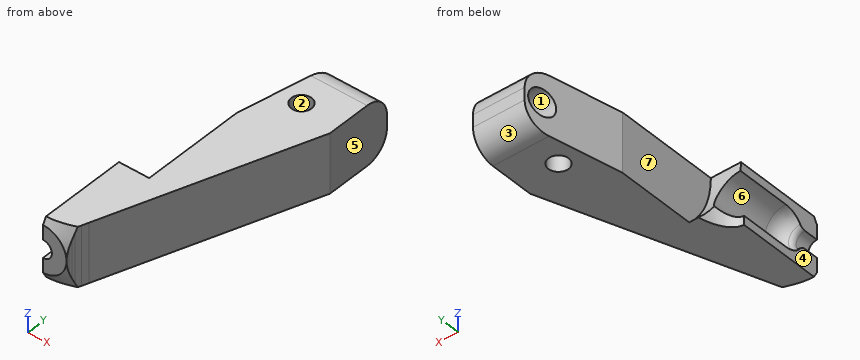
from build123d import *

# Parameters (mm, degrees)
SKETCH1_R                      = 3
BOSS_EXTRUDE2_DEPTH            = 17.7
CUT_EXTRUDE1_REACH             = 94.786
CUT_EXTRUDE1_DIRECTION_2_REACH = 94.786
SKETCH6_RX                     = 12.258033
SKETCH6_RY                     = 6.491927
CUT_EXTRUDE2_DEPTH             = 48.7
SKETCH7_R                      = 6.19409
CUT_EXTRUDE3_DEPTH             = 60.7
SKETCH8_R                      = 4
CUT_EXTRUDE4_DEPTH             = 48
FILLET1_R                      = 7
SKETCH10_OUTSIDE_W             = 249.546
SKETCH10_OUTSIDE_H             = 207.246
SKETCH10_OUTSIDE_R             = 7
CUT_EXTRUDE5_DEPTH             = 48
CUT_EXTRUDE5_TAPER             = 60
CUT_EXTRUDE8_DEPTH             = 44


with BuildPart() as part:
    # Sketch1 → Boss-Extrude2 (new body)
    with BuildSketch(Plane.XY):
        with BuildLine():
            Line((39, -51.503555), (34.837666, -51.503555))
            Line((34.837666, -51.503555), (25.162334, -51.503555))
            Line((25.162334, -51.503555), (21, -51.503555))
            Line((21, -51.503555), (21, -28.6))
            Line((21, -28.6), (15.376404, 0))
            Line((15.376404, 0), (0, 0))
            Line((0, 0), (0, -20.136364))
            Line((0, -20.136364), (21.048788, -80.412439))
            add(Edge.make_bspline(
                [(21.669142, -82.188906), (21.466678, -81.609123), (21.259066, -81.014599), (21.048788, -80.412439)],
                knots=[0.75, 0.75, 0.75, 0.75, 1, 1, 1, 1], degree=3))
            add(Edge.make_bspline(
                [(22.255532, -83.868113), (22.06924, -83.334643), (21.871606, -82.768689), (21.669142, -82.188906)],
                knots=[0.5, 0.5, 0.5, 0.5, 0.75, 0.75, 0.75, 0.75], degree=3))
            add(Edge.make_bspline(
                [(22.524034, -84.637007), (22.439154, -84.393941), (22.348677, -84.134848), (22.255532, -83.868113)],
                knots=[0.375, 0.375, 0.375, 0.375, 0.5, 0.5, 0.5, 0.5], degree=3))
            add(Edge.make_bspline(
                [(22.758263, -85.307753), (22.688292, -85.107381), (22.608914, -84.880073), (22.524034, -84.637007)],
                knots=[0.25, 0.25, 0.25, 0.25, 0.375, 0.375, 0.375, 0.375], degree=3))
            add(Edge.make_bspline(
                [(22.855261, -85.585519), (22.825847, -85.50129), (22.793248, -85.407938), (22.758263, -85.307753)],
                knots=[0.1875, 0.1875, 0.1875, 0.1875, 0.25, 0.25, 0.25, 0.25], degree=3))
            add(Edge.make_bspline(
                [(22.932474, -85.806631), (22.910958, -85.745015), (22.884674, -85.669748), (22.855261, -85.585519)],
                knots=[0.125, 0.125, 0.125, 0.125, 0.1875, 0.1875, 0.1875, 0.1875], degree=3))
            add(Edge.make_bspline(
                [(23, -86), (22.975508, -85.929864), (22.932474, -85.806631)],
                knots=[0, 0, 0, 0.125, 0.125, 0.125], degree=2))
            Line((23, -86), (37, -86))
            add(Edge.make_bspline(
                [(37.068167, -85.804796), (37.025162, -85.927946), (37, -86)],
                knots=[0.875, 0.875, 0.875, 1, 1, 1], degree=2))
            add(Edge.make_bspline(
                [(37.242328, -85.306061), (37.171936, -85.507639), (37.111171, -85.681646), (37.068167, -85.804796)],
                knots=[0.75, 0.75, 0.75, 0.75, 0.875, 0.875, 0.875, 0.875], degree=3))
            add(Edge.make_bspline(
                [(37.47673, -84.63482), (37.392157, -84.877005), (37.31272, -85.104482), (37.242328, -85.306061)],
                knots=[0.625, 0.625, 0.625, 0.625, 0.75, 0.75, 0.75, 0.75], degree=3))
            add(Edge.make_bspline(
                [(37.744144, -83.869041), (37.651111, -84.135454), (37.561302, -84.392634), (37.47673, -84.63482)],
                knots=[0.5, 0.5, 0.5, 0.5, 0.625, 0.625, 0.625, 0.625], degree=3))
            add(Edge.make_bspline(
                [(38.330881, -82.18884), (38.128355, -82.768803), (37.930211, -83.336215), (37.744144, -83.869041)],
                knots=[0.25, 0.25, 0.25, 0.25, 0.5, 0.5, 0.5, 0.5], degree=3))
            add(Edge.make_bspline(
                [(38.951212, -80.412439), (38.741, -81.014409), (38.533408, -81.608878), (38.330881, -82.18884)],
                knots=[0, 0, 0, 0, 0.25, 0.25, 0.25, 0.25], degree=3))
            Line((38.951212, -80.412439), (60, -20.136364))
            Line((60, -20.136364), (60, 0))
            Line((60, 0), (44.6, 0))
            Line((44.6, 0), (39, -28))
            Line((39, -28), (39, -51.503555))
        make_face()
        with Locations((48, -16)):
            Circle(SKETCH1_R, mode=Mode.SUBTRACT)
        with Locations((12, -16)):
            Circle(SKETCH1_R, mode=Mode.SUBTRACT)
    extrude(amount=BOSS_EXTRUDE2_DEPTH)

    # Sketch2 → Cut-Revolve2 (revolve, cut)
    with BuildSketch(Plane.ZY.offset(-30), mode=Mode.PRIVATE) as cut_revolve2_sk:
        with BuildLine():
            ThreePointArc((11.5, -81.75), (11.729241, -80.820262), (12.364412, -80.103659))
            ThreePointArc((12.364412, -80.103659), (14.333443, -77.882187), (15.04409, -75))
            Line((15.04409, -75), (15.04409, -57.48))
            Line((15.04409, -57.48), (8.85, -57.48))
            Line((8.85, -57.48), (8.85, -86))
            Line((8.85, -86), (11.5, -86))
            Line((11.5, -86), (11.5, -81.75))
        make_face()
    revolve(cut_revolve2_sk.sketch.rotate(Axis((30, -86, 8.85), (0, 1, 0)), 180), axis=Axis((30, -86, 8.85), (0, 1, 0)), mode=Mode.SUBTRACT)

    # Cut-Extrude1: up to this face of the body (flat: up to its plane)
    cut_extrude1_end = Plane(part.part.faces().sort_by_distance((39, -39.751777, 8.85))[0])
    # Sketch3 → Cut-Extrude1 (cut, up to the picked face)
    with BuildSketch(Plane.ZY.offset(-30), mode=Mode.PRIVATE) as cut_extrude1_sk1:
        with BuildLine():
            Line((0, -51.503555), (17.7, -51.503555))
            Line((17.7, -51.503555), (17.7, -59.152297))
            add(Edge.make_bspline(
                [(17.7, -59.152297), (7.335394, -59.008853), (0, -51.503555)],
                knots=[0, 0, 0, 1, 1, 1], degree=2))
        make_face()
    cut_extrude1_tool1 = split(extrude(cut_extrude1_sk1.sketch, amount=-CUT_EXTRUDE1_REACH, mode=Mode.PRIVATE), bisect_by=cut_extrude1_end, keep=Keep.BOTH, mode=Mode.PRIVATE)
    add(cut_extrude1_tool1.solids().sort_by(Axis((30, -54.604638, 10.907898), (1, 0, 0)))[0], mode=Mode.SUBTRACT)

    # Cut-Extrude1 direction 2: up to this face of the body (flat: up to its plane)
    cut_extrude1_direction_2_end = Plane(part.part.faces().sort_by_distance((21, -40.051777, 8.85))[0])
    # Sketch3 → Cut-Extrude1 direction 2 (cut, up to the picked face)
    with BuildSketch(Plane.ZY.offset(-30), mode=Mode.PRIVATE) as cut_extrude1_direction_2_sk1:
        with BuildLine():
            Line((0, -51.503555), (17.7, -51.503555))
            Line((17.7, -51.503555), (17.7, -59.152297))
            add(Edge.make_bspline(
                [(17.7, -59.152297), (7.335394, -59.008853), (0, -51.503555)],
                knots=[0, 0, 0, 1, 1, 1], degree=2))
        make_face()
    cut_extrude1_direction_2_tool1 = split(extrude(cut_extrude1_direction_2_sk1.sketch, amount=CUT_EXTRUDE1_DIRECTION_2_REACH, mode=Mode.PRIVATE), bisect_by=cut_extrude1_direction_2_end, keep=Keep.BOTH, mode=Mode.PRIVATE)
    add(cut_extrude1_direction_2_tool1.solids().sort_by(Axis((30, -54.604638, 10.907898), (-1, 0, 0)))[0], mode=Mode.SUBTRACT)

    # Sketch6 → Cut-Extrude2 (cut)
    with BuildSketch(Plane(origin=(0, 0, 8.85), x_dir=(-1, 0, 0), z_dir=(0, 0, -1))):
        with Locations(Location((-30, -47.968312), (0, 0, 90))):
            Ellipse(SKETCH6_RX, SKETCH6_RY)
    extrude(amount=CUT_EXTRUDE2_DEPTH, mode=Mode.SUBTRACT)

    # Sketch7 → Cut-Extrude3 (cut)
    with BuildSketch(Plane(origin=(0, 0, 0), x_dir=(1, 0, 0), z_dir=(0, 1, 0))):
        with Locations(Location((30, -8.85, 0), (0, 0, 90))):
            Circle(SKETCH7_R)
    extrude(amount=-CUT_EXTRUDE3_DEPTH, mode=Mode.SUBTRACT)

    # Sketch8 → Cut-Extrude4 (cut)
    with BuildSketch(Plane.ZY.offset(-6)):
        with Locations((8.85, -5)):
            Circle(SKETCH8_R)
    extrude(amount=-CUT_EXTRUDE4_DEPTH, mode=Mode.SUBTRACT)

    # Fillet1
    fillet1_edges = [part.edges().sort_by_distance(p)[0] for p in [
        (7.688202, 0, 17.7),
        (52.3, 0, 0),
        (7.688202, 0, 0),
        (52.3, 0, 17.7),
    ]]
    fillet(fillet1_edges, radius=FILLET1_R)

    # Sketch10 outside → Cut-Extrude5 (cut)
    with BuildSketch(Plane.XZ.offset(86)):
        with Locations((30, 8.85)):
            Rectangle(SKETCH10_OUTSIDE_W, SKETCH10_OUTSIDE_H)
        with Locations((30, 8.85)):
            Circle(SKETCH10_OUTSIDE_R, mode=Mode.SUBTRACT)
    extrude(amount=-CUT_EXTRUDE5_DEPTH, taper=CUT_EXTRUDE5_TAPER, mode=Mode.SUBTRACT)

    # Sketch12 → Cut-Extrude8 (cut)
    with BuildSketch(Plane.XY.offset(17.7)):
        Polygon((30, -86), (30, 13.730719), (-24.441977, 10.861444), (-8.282064, -99.477746), align=None)
    extrude(amount=-CUT_EXTRUDE8_DEPTH, mode=Mode.SUBTRACT)


solid = part.part
Model file for the job. Use its own axes, mm. Face numbers are marked on the shaded views. A direction names the side the tool comes from. Coordinates: 2 decimals unless noted, no trailing zeros. Order: outer loops, then holes, each group sorted by start corner. A loop starts at its lowest first (then second) coordinate and runs counter-clockwise, first axis right, second up. Notation, with made-up numbers: M 13,-4.75 L 20,-4.75 A33 cw 20,34.25 Z; hole C 30.25,46.5 d8. An arc over 180 degrees is marked long. Return JSON: item names as keys, results as strings.
1. Flat gauge pins, fed straight in: pin 1 (4 mm diameter, centred on y = -7, z = 11, fed in from -X); pin 2 (7 mm diameter, centred on y = -5, z = 8.85, fed in from -X); pin 3 (10 mm diameter, centred on x = 51.5, y = -48, fed in from +Z); pin 4 (1 mm diameter, centred on x = 43, z = 9.5, fed in from +Y). Where does each tip first touch, or does it go through?
Ans:
{"pin 1": "x = 42.8", "pin 2": "x = 54", "pin 3": "z = 17.7", "pin 4": "y = -8.83"}
2. Saw through at D-D (y = -5). Give the cut face in (x, z), and give its area (3 significant figures).
Ans:
{"outline": "M 43.6,0.29 L 60,0.29 L 60,17.41 L 43.6,17.41 L 43.6,12.85 L 54,12.85 L 54,4.85 L 43.6,4.85 Z", "area": "198 mm^2"}
3. Saw through at B-B (y = -16). Give the cut face in (x, z).
Ans:
{"outline": "M 41.4,0 L 45,0 L 45,17.7 L 41.4,17.7 Z; M 51,0 L 60,0 L 60,17.7 L 51,17.7 Z"}
4. Tool access for the marked faces 5, 6 and 7: list every direction of +Z, -Z, +X, -X, +Y, -Y with a clear straight run to the whole face (end or side of a thin tool).
Ans:
{"face 5": "+Z, -Z, +X, +Y, -Y", "face 6": "-X, +Y", "face 7": "+Z, -X, +Y"}
5. Pull direction Y, two halves, no side cores. Call the marked faces 1, 2, 3 and 4: +Y half, -Y half, draft (parallel to the pull), parting line (faces both ways), or undercut.
Ans:
{"face 1": "undercut", "face 2": "undercut", "face 3": "+Y half", "face 4": "draft"}
6. Drill centre lines: probe 1 along Z at (x, y) = (48, -4); probe 2 along X at (y, z) = (-14.5, 9.25); probe 3 along X at (y, z) = (-17, 7). Where is each one in solid material? Low to high.
Ans:
{"probe 1": "0.68 to 4.98, 12.72 to 17.02", "probe 2": "41.7 to 45.4, 50.6 to 60", "probe 3": "41.2 to 45.17, 50.83 to 60"}
7. Saw through at C-C (x = 52.5). Give the cut face in (y, z).
Ans:
{"outline": "M -41.61,0 L -7,0 A7 ccw 0,7 L 0,10.7 A7 ccw -7,17.7 L -41.61,17.7 Z; hole C -5,8.85 d8"}
8. Saw through at A-A (x = 48). Give the cut face in (y, z), and give its area (3 significant figures).
Ans:
{"outline": "M -54.5,0 L -19,0 L -19,17.7 L -54.5,17.7 Z; M -13,0 L -7,0 A7 ccw 0,7 L 0,10.7 A7 ccw -7,17.7 L -13,17.7 Z; hole C -5,8.85 d8", "area": "787 mm^2"}
